Design review of the part built by this model. Coordinates are the model's own, in mm. Face numbers are marked on the shaded views. A direction names the side the tool comes from. Coordinates: 2 decimals unless noted, no trailing zeros. Write each loop counter-clockwise with the first axis right and the second up, starting at its lowest first coordinate (ties: lowest second). Pieces come first, ordered by that corner, then holes.
Q1. Mouldability with a two-part tool opening along X and no side actions: class the marked faces 1, 2 and 3 as pulls with the +X half, pulls with the -X half, needs draft (parallel to the pull), parting line crosses it, or undercut.
Q2. Machinability: for the marked faces 4 and 5, which of the approach directions +Z, -Z, +X, -X, +Y, -Y give a long, thin tool a straight path to every point of the face, cutting with its end or side? Answer none if there is none.
Q3. For probe 1 along X at (y, z) = (50.5, 78); probe 2 along X at (y, z) = (58.5, 107); probe 3 along Z at (x, y) = (-28, 59), list the stretches that pass through material, from the lowest coordinate up.
Q4. Take a section at D-D (y = 74). Give the boundary of the cut face in (x, z), and give its area (3 significant figures).
Q5. Take a section at A-A (y = 62). State how many separate pieces and enclosed holes the cut face has, and give its area (3 significant figures).
Q6. Insertion check: pin 1 (8 mm diameter, centred on y = 69.5, z = -69, fed in from +X); pin 2 (4 mm diameter, centred on x = -68.5, y = 59.5, fed in from -Z); pin 3 (5.5 mm diameter, centred on x = -8.5, y = 59.5, fed in from -Z); pin 4 (17.5 mm diameter, centred on x = -41.5, z = 78, fed in from +Y). Each pin has a flat end and moves straight along its axis. Give the tip position at first contact, or say it passes through.
Q7. Take a section at B-B (z = -107). Give the boundary of the cut face in (x, y), and give its area (3 significant figures).
Q8. Take a section at C-C (x = -8). Give the boundary of the cut face in (y, z), and give its area (3 significant figures).
```python
from build123d import *

# Parameters (mm, degrees)
SIDE_WALL_DEPTH           = 5
END_FLANGE_A_DEPTH        = 50
FLANGE_A_POCKET_DEPTH     = 15
ARCH_SHELL_DEPTH          = 75
SIDE_START                = -5
SIDE_WALL_EXTENSION_DEPTH = 5
FLANGE_START              = -75
FLANGE_A_RIM_DEPTH        = 75
END_FLANGE_B_SKETCH_W     = 75
END_FLANGE_B_SKETCH_H     = 20
END_FLANGE_B_DEPTH        = 50
FLANGE_B_POCKET_DEPTH     = 15
FLANGE_B_RIM_DEPTH        = 75
BOLT_HOLES_SKETCH_R       = 4
BOLT_HOLES_4X_DEPTH       = 75
CORNER_FILLETS_R10_A_R    = 10
CORNER_FILLETS_R10_B_R    = 10
CORNER_FILLETS_R10_C_R    = 10
CORNER_FILLETS_R10_D_R    = 10


with BuildPart() as part:
    # Side Wall Profile Sketch → Side Wall (new body)
    with BuildSketch(Plane(origin=(0, 0, 0), x_dir=(0, 0, -1), z_dir=(1, 0, 0))):
        with BuildLine():
            ThreePointArc((56.118661154, 45.107603243), (0, 72), (-56.118661154, 45.107603243))
            Line((-56.118661154, 45.107603243), (-115, 45.107603243))
            Line((-115, 45.107603243), (-115, 65.107603243))
            Line((-115, 65.107603243), (-65, 65.107603243))
            ThreePointArc((-65, 65.107603243), (0, 92), (65, 65.107603243))
            Line((65, 65.107603243), (115, 65.107603243))
            Line((115, 65.107603243), (115, 45.107603243))
            Line((115, 45.107603243), (95, 45.107603243))
            Line((95, 45.107603243), (56.118661154, 45.107603243))
        make_face()
    extrude(amount=-SIDE_WALL_DEPTH)

    # End Flange A Sketch → End Flange A (add)
    with BuildSketch(Plane.XY.offset(115)):
        Polygon((0, 45.107603243), (-75, 45.107603243), (-75, 65.107603243), (-5, 65.107603243), (0, 65.107603243), align=None)
    extrude(amount=-END_FLANGE_A_DEPTH)

    # Flange A Pocket Sketch → Flange A Pocket (cut)
    with BuildSketch(Plane(origin=(0, 65.107603243, 0), x_dir=(1, 0, 0), z_dir=(0, 1, 0))):
        Polygon((-10, -90), (-5, -90), (-5, -65), (-70, -65), (-70, -90), (-65, -90), (-54, -110), (-21, -110), align=None)
    extrude(amount=-FLANGE_A_POCKET_DEPTH, mode=Mode.SUBTRACT)

    # Arch Shell Sketch → Arch Shell (add)
    with BuildSketch(Plane(origin=(0, 0, 0), x_dir=(0, 0, -1), z_dir=(1, 0, 0))):
        with BuildLine():
            Line((-56.118661154, 45.107603243), (-55.986211495, 45.107603243))
            ThreePointArc((-55.986211495, 45.107603243), (0, 71.896813197), (55.986211495, 45.107603243))
            Line((55.986211495, 45.107603243), (56.118661154, 45.107603243))
            ThreePointArc((56.118661154, 45.107603243), (0, 72), (-56.118661154, 45.107603243))
        make_face()
    extrude(amount=-ARCH_SHELL_DEPTH)

    # Side Wall Extension Sketch → Side Wall Extension (add)
    with BuildSketch(Plane.ZY.offset(75).offset(SIDE_START)):
        with BuildLine():
            ThreePointArc((-65, 65.043834782), (-73.247030889, 55.592921393), (-80.131171043, 45.107603243))
            Line((-80.131171043, 45.107603243), (-65, 45.107603243))
            Line((-65, 45.107603243), (-56.118661154, 45.107603243))
            ThreePointArc((-56.118661154, 45.107603243), (0, 72), (56.118661154, 45.107603243))
            Line((56.118661154, 45.107603243), (65, 45.107603243))
            Line((65, 45.107603243), (65, 65.043834782))
            ThreePointArc((65, 65.043834782), (0, 91.95488265), (-65, 65.043834782))
        make_face()
    extrude(amount=SIDE_WALL_EXTENSION_DEPTH)

    # Flange A Rim Sketch → Flange A Rim (add)
    with BuildSketch(Plane.ZY.offset(75).offset(FLANGE_START)):
        with BuildLine():
            Line((55.986211495, 45.107603243), (65, 45.107603243))
            Line((65, 45.107603243), (65, 50.107603243))
            Line((65, 50.107603243), (51.559478713, 50.107603243))
            ThreePointArc((51.559478713, 50.107603243), (53.830928569, 47.659027238), (55.986211495, 45.107603243))
        make_face()
    extrude(amount=FLANGE_A_RIM_DEPTH)

    # End Flange B Sketch → End Flange B (add)
    with BuildSketch(Plane(origin=(0, 0, -115), x_dir=(-1, 0, 0), z_dir=(0, 0, -1))):
        with Locations((37.5, 55.107603243)):
            Rectangle(END_FLANGE_B_SKETCH_W, END_FLANGE_B_SKETCH_H)
    extrude(amount=-END_FLANGE_B_DEPTH)

    # Flange B Pocket Sketch → Flange B Pocket (cut)
    with BuildSketch(Plane(origin=(0, 65.107603243, 0), x_dir=(1, 0, 0), z_dir=(0, 1, 0))):
        Polygon((-56.25, 110), (-70, 90), (-70, 65), (-5, 65), (-5, 90), (-18.75, 110), (-37.5, 110), align=None)
    extrude(amount=-FLANGE_B_POCKET_DEPTH, mode=Mode.SUBTRACT)

    # Flange B Rim Sketch → Flange B Rim (add)
    with BuildSketch(Plane(origin=(0, 0, 0), x_dir=(0, 0, -1), z_dir=(1, 0, 0))):
        with BuildLine():
            Line((65, 45.107603243), (65, 50.107603243))
            Line((65, 50.107603243), (51.559478713, 50.107603243))
            ThreePointArc((51.559478713, 50.107603243), (53.830928569, 47.659027238), (55.986211495, 45.107603243))
            Line((55.986211495, 45.107603243), (65, 45.107603243))
        make_face()
    extrude(amount=-FLANGE_B_RIM_DEPTH)

    # Bolt Holes Sketch → Bolt Holes 4x (cut)
    with BuildSketch(Plane(origin=(0, 65.107603243, 0), x_dir=(1, 0, 0), z_dir=(0, 1, 0))):
        with Locations(Location((-8, 107, 0), (0, 0, 270))):
            Circle(BOLT_HOLES_SKETCH_R)
        with Locations(Location((-67, 107, 0), (0, 0, 270))):
            Circle(BOLT_HOLES_SKETCH_R)
        with Locations(Location((-8, -107, 0), (0, 0, 270))):
            Circle(BOLT_HOLES_SKETCH_R)
        with Locations(Location((-67, -107, 0), (0, 0, 270))):
            Circle(BOLT_HOLES_SKETCH_R)
    extrude(amount=-BOLT_HOLES_4X_DEPTH, mode=Mode.SUBTRACT)

    # Corner Fillets R10 A
    corner_fillets_r10_a_edges = [part.edges().sort_by_distance(p)[0] for p in [
        (0, 55.107603243, 115),
    ]]
    fillet(corner_fillets_r10_a_edges, radius=CORNER_FILLETS_R10_A_R)

    # Corner Fillets R10 B
    corner_fillets_r10_b_edges = [part.edges().sort_by_distance(p)[0] for p in [
        (-75, 55.107603243, 115),
    ]]
    fillet(corner_fillets_r10_b_edges, radius=CORNER_FILLETS_R10_B_R)

    # Corner Fillets R10 C
    corner_fillets_r10_c_edges = [part.edges().sort_by_distance(p)[0] for p in [
        (-75, 55.107603243, -115),
    ]]
    fillet(corner_fillets_r10_c_edges, radius=CORNER_FILLETS_R10_C_R)

    # Corner Fillets R10 D
    corner_fillets_r10_d_edges = [part.edges().sort_by_distance(p)[0] for p in [
        (0, 55.107603243, -115),
    ]]
    fillet(corner_fillets_r10_d_edges, radius=CORNER_FILLETS_R10_D_R)


solid = part.part
```
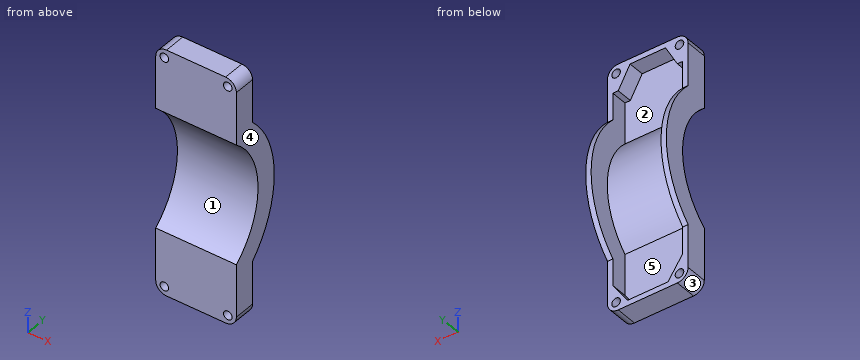
Response:
1. face 1: needs draft
1. face 2: undercut
1. face 3: pulls with the -X half
2. face 4: +Z, -Z, +X, +Y, -Y
2. face 5: +Y
3. probe 1: x = -75 to -70, -5 to 0
3. probe 2: x = -74.8 to -71, -63 to -55.65, -19.35 to -12, -4 to -0.2
3. probe 3: z = -115 to -110, -41.27 to -41.09, 41.09 to 41.27, 110 to 115
4. outline: (-75, -54.59) - (-70, -54.59) - (-70, 54.59) - (-75, 54.59) - close; (-5, -54.66) - (0, -54.66) - (0, 54.66) - (-5, 54.66) - close
4. area: 1,090 mm2
5. separate pieces: 2
5. enclosed holes: 6
5. area: 2,660 mm2
6. pin 1: passes through
6. pin 2: stops at z = -114.89
6. pin 3: stops at z = -115
6. pin 4: stops at y = 50.11
7. outline: (-74.8, 45.11) - (-71, 45.11) - (-71, 65.11) - (-74.8, 65.11) - close; (-63, 45.11) - (-12, 45.11) - (-12, 65.11) - (-16.69, 65.11) - (-16.69, 50.11) - (-58.31, 50.11) - (-58.31, 65.11) - (-63, 65.11) - close; (-4, 45.11) - (-0.2, 45.11) - (-0.2, 65.11) - (-4, 65.11) - close
7. area: 548 mm2
8. outline: (45.11, -114.8) - (65.11, -114.8) - (65.11, -111) - (45.11, -111) - close; (45.11, -103) - (65.11, -103) - (65.11, -94.36) - (50.11, -94.36) - (50.11, -51.7) arc R72 ccw to (50.11, 51.7) - (50.11, 90) - (65.11, 90) - (65.11, 103) - (45.11, 103) - (45.11, 55.99) arc R71.9 cw to (45.11, -55.99) - close; (45.11, 111) - (65.11, 111) - (65.11, 114.8) - (45.11, 114.8) - close
8. area: 980 mm2
